from build123d import *

# Parameters (mm, degrees)
BASE_DISC_SKETCH_R          = 55
BASE_DISC_SKETCH_R_2        = 16
BASE_DISC_110_BORE_32_DEPTH = 10
TOP_RAILS_SKETCH_W          = 12
TOP_RAILS_SKETCH_H          = 94.678403028
TOP_RAILS_DEPTH             = 20
BOTTOM_LEGS_SKETCH_W        = 94.678403028
BOTTOM_LEGS_SKETCH_H        = 12
BOTTOM_LEGS_DEPTH           = 20


with BuildPart() as part:
    # Base Disc Sketch → Base Disc Ø110 Bore Ø32 (new body)
    with BuildSketch(Plane(origin=(0, 0, 0), x_dir=(1, 0, 0), z_dir=(0, 1, 0))):
        with Locations(Location((0, 0, 0), (0, 0, 270))):
            Circle(BASE_DISC_SKETCH_R)
        with Locations(Location((0, 0, 0), (0, 0, 270))):
            Circle(BASE_DISC_SKETCH_R_2, mode=Mode.SUBTRACT)
    extrude(amount=BASE_DISC_110_BORE_32_DEPTH)

    # Top Rails Sketch → Top Rails (add)
    with BuildSketch(Plane(origin=(0, 10, 0), x_dir=(1, 0, 0), z_dir=(0, 1, 0))):
        with Locations((22, 0)):
            Rectangle(TOP_RAILS_SKETCH_W, TOP_RAILS_SKETCH_H)
        with Locations((-22, 0)):
            Rectangle(TOP_RAILS_SKETCH_W, TOP_RAILS_SKETCH_H)
    extrude(amount=TOP_RAILS_DEPTH)

    # Bottom Legs Sketch → Bottom Legs (add)
    with BuildSketch(Plane.XZ):
        with Locations((0, 22)):
            Rectangle(BOTTOM_LEGS_SKETCH_W, BOTTOM_LEGS_SKETCH_H)
        with Locations((0, -22)):
            Rectangle(BOTTOM_LEGS_SKETCH_W, BOTTOM_LEGS_SKETCH_H)
    extrude(amount=BOTTOM_LEGS_DEPTH)


solid = part.part
Verification items for the finished model (mm, model axes). A direction names the side the tool comes from. Coordinates: 2 decimals unless noted, no trailing zeros. Loops run counter-clockwise (first coordinate to the right, second up) from the corner with the lowest first, then second, coordinate; pieces in that order, holes last. Notation, with made-up numbers: M -5,-3.75 L 2,-3.75 A17 cw 2,17.25 Z; hole C 89.25,1 d3. An arc over 180 degrees is marked long. One line per item, written item: value.
1. Gauge pin test, flat ends, axial feed: P1, Ø16, axis at x = 3.5, y = -10.5, coming from the -Z side; P2, Ø9.5, axis at x = 19.5, y = 24, coming from the +Z side; P3, Ø9.5, axis at y = -8, z = -20.5, coming from the -X side. Record the tip position at first contact, or that the pin passes through.
Answers follow:
P1: z = -28
P2: z = 47.34
P3: x = -47.34
2. Section check A-A on y = -11. Record the cut outline in (x, z).
Answers follow:
outline: M -47.34,-28 L 47.34,-28 L 47.34,-16 L -47.34,-16 Z; M -47.34,16 L 47.34,16 L 47.34,28 L -47.34,28 Z
3. Mould release check, pull along X, two halves, no side actions. Record for faces 1 (the flat face through (-16, 20, 1)), 2 (the flat face through (47.339, -10, -22)), 3 (the flat face through (39, 10, -1)): pulls with the +X half, pulls with the -X half, needs draft (parallel to the pull), parting line crosses it, or undercut.
Answers follow:
face 1: undercut
face 2: pulls with the +X half
face 3: needs draft
4. Section check D-D on z = 40. Record the cut outline in (x, y).
Answers follow:
outline: M -37.75,0 L 37.75,0 L 37.75,10 L 28,10 L 28,30 L 16,30 L 16,10 L -16,10 L -16,30 L -28,30 L -28,10 L -37.75,10 Z
5. Section check B-B on z = -3. Record the cut outline in (x, y), plus the area to 3 significant figures.
Answers follow:
outline: M -54.92,0 L -15.72,0 L -15.72,10 L -16,10 L -16,30 L -28,30 L -28,10 L -54.92,10 Z; M 15.72,0 L 54.92,0 L 54.92,10 L 28,10 L 28,30 L 16,30 L 16,10 L 15.72,10 Z
area: 1,260 mm^2
6. Section check C-C on x = -24. Record the cut outline in (y, z), plus the area to 3 significant figures.
Answers follow:
outline: M -20,-28 L 0,-28 L 0,-49.49 L 10,-49.49 L 10,-47.34 L 30,-47.34 L 30,47.34 L 10,47.34 L 10,49.49 L 0,49.49 L 0,28 L -20,28 L -20,16 L 0,16 L 0,-16 L -20,-16 Z
area: 3,360 mm^2
7. Material ranges on line 1 along Z through (x, y) = (0, 3.5); line 2 along X through (y, z) = (27, 22.5), recorded low to high. Write a range as from..to.
Answers follow:
line 1: -55..-16, 16..55
line 2: -28..-16, 16..28
8. Set-up check for faces 4 (the flat face through (-38, 10, -1)), 5 (the flat face through (16, 20, 1)), 6 (the flat face through (-1, -10, -28)), 7 (the flat face through (1, 0, 38)), 8 (the flat face through (-47.339, -10, 22)): record each of +Z, -Z, +X, -X, +Y, -Y from which the full face is reachable in a straight line by a thin tool's end or side.
Answers follow:
face 4: +Z, -Z, -X, +Y
face 5: +Z, -Z, +Y
face 6: -Z, +X, -X, -Y
face 7: +Z, +X, -X, -Y
face 8: +Z, -Z, -X, -Y
